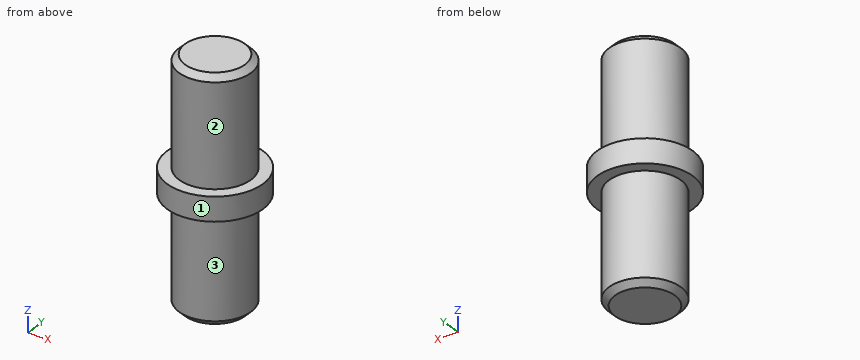
from build123d import *

# Parameters (mm, degrees)
SKETCH_1_R      = 4
EXTRUDE_1_DEPTH = 1
SKETCH_2_R      = 3
EXTRUDE_2_DEPTH = 9
CHAMFER_1_SIZE  = 0.5


with BuildPart() as part:
    # 草图1 → 凸台-拉伸1 (new, symmetric)
    with BuildSketch(Plane.XY):
        Circle(SKETCH_1_R)
    extrude(amount=EXTRUDE_1_DEPTH, both=True)

    # 草图2 → 凸台-拉伸2 (add)
    with BuildSketch(Plane.XY.offset(1)):
        Circle(SKETCH_2_R)
    extrude_2 = extrude(amount=EXTRUDE_2_DEPTH)

    # 镜向5: 凸台-拉伸2 across plane
    add(extrude_2.mirror(Plane.XY))

    # 倒角1
    chamfer_1_edges = [part.edges().sort_by_distance(p)[0] for p in [
        (-3, 0, -10),
        (-3, 0, 10),
    ]]
    chamfer(chamfer_1_edges, length=CHAMFER_1_SIZE)


solid = part.part
Work out the finished part from the listing and answer in its coordinate system (mm). Face numbers are marked on the shaded views. A direction names the side the tool comes from. Round coordinates to 2 decimals unless told otherwise and drop trailing zeros. Write each loop counter-clockwise with the first axis right and the second up, starting at its lowest first coordinate (ties: lowest second). Pieces come first, ordered by that corner, then holes. Notation, with made-up numbers: (79, 70) - (117, 70) arc R9 cw to (117, 82) - close; hole circle Ø4 at (-5, 48.25). An arc over 180 degrees is marked (long way). Answer in a Markdown table with one row per item. Add a question column.
1. Given pin 1 (2 mm diameter, centred on x = 2.5, z = 3, fed in from +Y); pin 2 (3 mm diameter, centred on x = 0.5, y = -2.5, fed in from +Z); pin 3 (2 mm diameter, centred on x = 2.5, y = -3, fed in from -Z); pin 4 (2 mm diameter, centred on y = 3, z = 1, fed in from +X), each flat-ended and moving along its own axis, determine where each tip first touches the part or whether it passes through.
2. A cutting plane is placed at A-A, the plane x = 0. Determine the outline of the cut face in (y, z), and give its area (4 significant figures).
3. A cutting plane is placed at B-B, the plane z = 0.5. Determine the outline of the cut face in (x, y).
4. Find the intervals of material crossed by line 1 along Z through (x, y) = (-2.5, -2.75); line 2 along Z through (x, y) = (2.75, -1); line 3 along Y through (x, z) = (0.25, -1.75), in increasing order. Write a range as from..to.
5. A cutting plane is placed at D-D, the plane x = -3.5. Determine the outline of the cut face in (y, z).
6. For the marked faces 1, 2 and 3, determine the directions among +Z, -Z, +X, -X, +Y, -Y from which every point of the face is accessible in a straight line to the end or side of a thin tool.
7. A cutting plane is placed at C-C, the plane z = -3.5. Determine the outline of the cut face in (x, y).
Worked out:
| question | item | result |
|---|---|---|
| 1 | pin 1 | y = 2.6 |
| 1 | pin 2 | z = 10 |
| 1 | pin 3 | z = -9.59 |
| 1 | pin 4 | x = 3.46 |
| 2 | outline | (-4, -1) - (-3, -1) - (-3, -9.5) - (-2.5, -10) - (2.5, -10) - (3, -9.5) - (3, -1) - (4, -1) - (4, 1) - (3, 1) - (3, 9.5) - (2.5, 10) - (-2.5, 10) - (-3, 9.5) - (-3, 1) - (-4, 1) - close |
| 2 | area | 123.5 mm^2 |
| 3 | outline | circle Ø8 at (0, 0) |
| 4 | line 1 | -1..1 |
| 4 | line 2 | -9.57..9.57 |
| 4 | line 3 | -2.99..2.99 |
| 5 | outline | (-1.94, -1) - (1.94, -1) - (1.94, 1) - (-1.94, 1) - close |
| 6 | face 1 | +Z, -Z |
| 6 | face 2 | +Z |
| 6 | face 3 | -Z |
| 7 | outline | circle Ø6 at (0, 0) |
